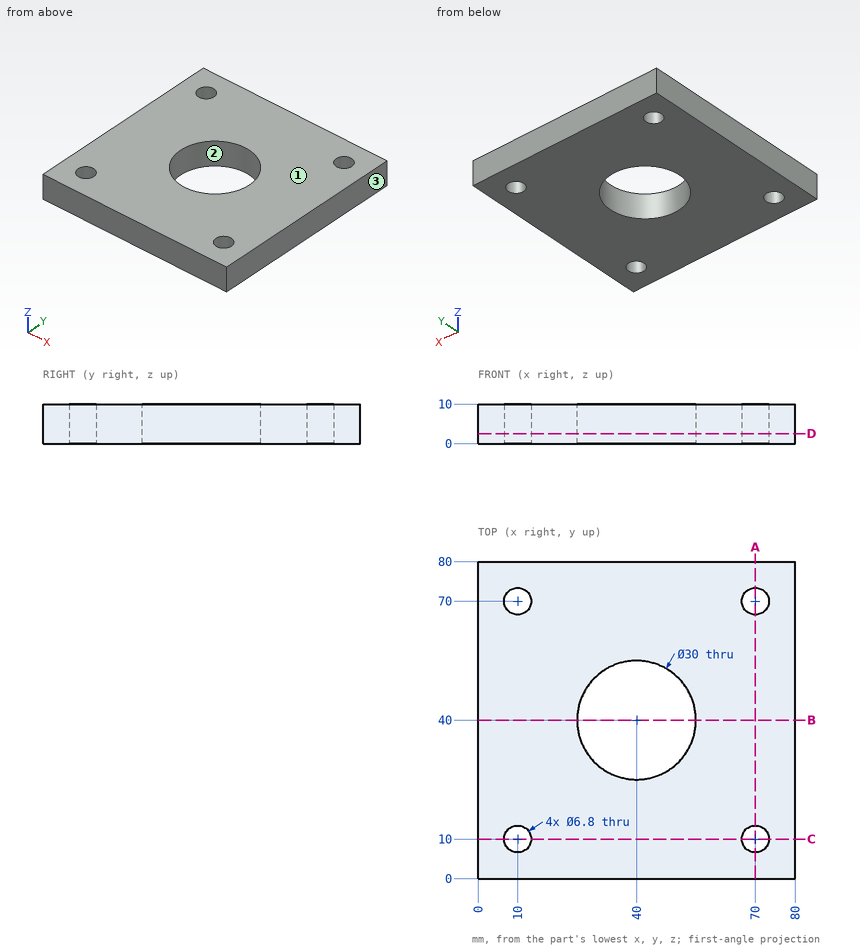
Study the drawing (mm; zero at the part's minimum x, y, z) and answer. Give positions to 0.01 mm unless a question says otherwise; leave off trailing zeros. Order: outer loops, then holes, each group sorted by start corner. A loop starts at its lowest first (then second) coordinate and runs counter-clockwise, first axis right, second up. Notation, with made-up numbers: (61, 47) - (84, 47) arc R33 cw to (84, 78) - close; hole circle Ø11 at (71.5, 37.5). An arc over 180 degrees is marked (long way). Answer as CSV lines item,"result". Start each with the question number.
Q1. The mould has two halves that part along X. Classify the marked faces 1, 2 and 3: +X half, -X half, draft (parallel to the pull), parting line (faces both ways), or undercut.
Q2. The part is cut by section B-B (y = 40). Write down the section's boundary in (x, z), then the cut area to 3 significant figures.
Q3. Find the intervals of material crossed by L1, parallel to Y at x = 7, z = 6; L2, parallel to Y at x = 70, z = 8.25; L3, parallel to X at y = 40.5, z = 5.25, in increasing order. Write a range as [from, to].
Q4. The part is cut by section D-D (z = 2.5). Write down the section's boundary in (x, y).
Q5. The part is cut by section A-A (x = 70). Write down the section's boundary in (y, z).
Check result:
1,face 1,"draft"
1,face 2,"undercut"
1,face 3,"+X half"
2,outline,"(0, 0) - (25, 0) - (25, 10) - (0, 10) - close; (55, 0) - (80, 0) - (80, 10) - (55, 10) - close"
2,area,"500 mm²"
3,L1,"y = [0, 8.4], [11.6, 68.4], [71.6, 80]"
3,L2,"y = [0, 6.6], [13.4, 66.6], [73.4, 80]"
3,L3,"x = [0, 25.01], [54.99, 80]"
4,outline,"(0, 0) - (80, 0) - (80, 80) - (0, 80) - close; hole circle Ø6.8 at (10, 10); hole circle Ø6.8 at (10, 70); hole circle Ø30 at (40, 40); hole circle Ø6.8 at (70, 10); hole circle Ø6.8 at (70, 70)"
5,outline,"(0, 0) - (6.6, 0) - (6.6, 10) - (0, 10) - close; (13.4, 0) - (66.6, 0) - (66.6, 10) - (13.4, 10) - close; (73.4, 0) - (80, 0) - (80, 10) - (73.4, 10) - close"
